CAD build for the part. Positions are in the model's coordinates, mm. A direction names the side the tool comes from. Coordinates: 2 decimals unless noted, no trailing zeros. Loops run counter-clockwise (first coordinate to the right, second up) from the corner with the lowest first, then second, coordinate; pieces in that order, holes last. Notation, with made-up numbers: M 30,69.25 L 80,69.25 A9 ccw 80,81.25 Z; hole C -20,24 d7. An arc over 180 degrees is marked long. Answer as a JSON object with one key per item and string values. Group by question number.
```python
from build123d import *

# Parameters (mm, degrees)
SKETCH1_W                = 50
SKETCH1_H                = 100
BOSS_EXTRUDE1_DEPTH      = 10
CUT_EXTRUDE1_DEPTH       = 10
BOSS_EXTRUDE2_DEPTH      = 180
BOSS_EXTRUDE2_DEPTH_BACK = 10
SKETCH3_W                = 50
SKETCH3_H                = 10
CUT_EXTRUDE2_DEPTH       = 180


with BuildPart() as part:
    # Sketch1 → Boss-Extrude1 (new body)
    with BuildSketch(Plane.XY):
        Rectangle(SKETCH1_W, SKETCH1_H)
    extrude(amount=BOSS_EXTRUDE1_DEPTH)

    # Sketch2 → Cut-Extrude1 (cut)
    with BuildSketch(Plane.XY.offset(10)):
        with BuildLine():
            Line((0.5, -35), (-0.5, -35))
            ThreePointArc((-0.5, -35), (-3.681980515, -33.681980515), (-5, -30.5))
            Line((-5, -30.5), (-5, 30.5))
            ThreePointArc((-5, 30.5), (-3.681980515, 33.681980515), (-0.5, 35))
            Line((-0.5, 35), (0.5, 35))
            ThreePointArc((0.5, 35), (3.681980515, 33.681980515), (5, 30.5))
            Line((5, 30.5), (5, -30.5))
            ThreePointArc((5, -30.5), (3.681980515, -33.681980515), (0.5, -35))
        make_face()
    extrude(amount=-CUT_EXTRUDE1_DEPTH, mode=Mode.SUBTRACT)

    # Sketch3 → Boss-Extrude2 (add, two sides: drawn at the far end of the back side and taken through both)
    with BuildSketch(Plane(origin=(0, 0, 0), x_dir=(-1, 0, 0), z_dir=(0, 0, -1)).offset(-BOSS_EXTRUDE2_DEPTH_BACK)):
        with Locations((0, 50)):
            Rectangle(SKETCH3_W, SKETCH3_H)
    extrude(amount=BOSS_EXTRUDE2_DEPTH + BOSS_EXTRUDE2_DEPTH_BACK)

    # Sketch4 → Cut-Extrude2 (cut)
    with BuildSketch(Plane.XZ.offset(-45)):
        with BuildLine():
            Line((1.63487738, -153.842941115), (0.63487738, -153.842941115))
            ThreePointArc((0.63487738, -153.842941115), (-2.547103135, -152.52492163), (-3.86512262, -149.342941115))
            Line((-3.86512262, -149.342941115), (-3.86512262, -28.342941115))
            ThreePointArc((-3.86512262, -28.342941115), (-2.547103135, -25.160960599), (0.63487738, -23.842941115))
            Line((0.63487738, -23.842941115), (1.63487738, -23.842941115))
            ThreePointArc((1.63487738, -23.842941115), (4.816857896, -25.160960599), (6.13487738, -28.342941115))
            Line((6.13487738, -28.342941115), (6.13487738, -149.342941115))
            ThreePointArc((6.13487738, -149.342941115), (4.816857896, -152.52492163), (1.63487738, -153.842941115))
        make_face()
    extrude(amount=-CUT_EXTRUDE2_DEPTH, mode=Mode.SUBTRACT)


solid = part.part
```
Item 1: Drill centre lines: L1, parallel to Z at x = 13, y = 7; L2, parallel to Y at x = 7.5, z = -140. Where is each one in solid material? Low to high. Write a range as from..to.
Item 2: Slice it at A-A, the plane z = -60. Write the cut outline in (x, y).
Item 3: Slice it at D-D, the plane z = -10. Write the cut outline in (x, y), then the cut area to 3 significant figures.
Item 4: Pull direction X, two halves, no side cores. Call faces 1 (the flat face through (-5, 55, -84)), 2 (the flat face through (-25, 49, -64)), 3 (the cylindrical face through (4.782, 49.93, -25.126)): released by +X, released by -X, zero draft, split by the parting line, or undercut.
Item 5: Pin check, flat tips, straight feed: pin 1 (1.5 mm diameter, centred on x = 10.5, z = -88.5, fed in from -Y); pin 2 (1.5 mm diameter, centred on x = -6, y = -18.5, fed in from -Z); pin 3 (12 mm diameter, centred on y = 33.5, z = -31.5, fed in from +X). Stop position of each tip, or through.
Item 6: Tool access for faces 4 (the flat face through (5.2, -1.8, 0)), 5 (the flat face through (-6, 3, 10)), 6 (the flat face through (6.135, 50, -88)), 7 (the cylindrical face through (-3.647, -33.717, 5.07)): list every direction of +Z, -Z, +X, -X, +Y, -Y with a clear straight run to the whole face (end or side of a thin tool).
Item 7: Slice it at B-B, the plane y = 26.5. Write the cut outline in (x, z), then the cut area to 3 significant figures.
Item 8: Slice it at C-C, the plane x = 19. Write the cut outline in (y, z).
Computed:
{
 "1": {"L1": "0..10", "L2": "45..55"},
 "2": {"outline": "M -25,45 L -3.87,45 L -3.87,55 L -25,55 Z; M 6.13,45 L 25,45 L 25,55 L 6.13,55 Z"},
 "3": {"outline": "M -25,45 L 25,45 L 25,55 L -25,55 Z", "area": "500 mm2"},
 "4": {"face 1": "zero draft", "face 2": "released by -X", "face 3": "undercut"},
 "5": {"pin 1": "y = 45", "pin 2": "z = 0", "pin 3": "through"},
 "6": {"face 4": "-Z, +X, -X, -Y", "face 5": "+Z, +X, -X, +Y, -Y", "face 6": "+Y, -Y", "face 7": "+Z, -Z"},
 "7": {"outline": "M -25,0 L -5,0 L -5,10 L -25,10 Z; M 5,0 L 25,0 L 25,10 L 5,10 Z", "area": "400 mm2"},
 "8": {"outline": "M -50,0 L 45,0 L 45,-180 L 55,-180 L 55,10 L -50,10 Z"}
}
